```python
from build123d import *

# Parameters (mm, degrees)
BOSS_EXTRUDE1_DEPTH      = 5.5
BOSS_EXTRUDE1_DEPTH_BACK = 5.5
SKETCH2_W                = 108
SKETCH2_H                = 22
CUT_EXTRUDE1_DEPTH       = 11
SKETCH4_W                = 9
SKETCH4_H                = 10
CUT_EXTRUDE2_DEPTH       = 11


with BuildPart() as part:
    # Sketch1 → Boss-Extrude1 (new, two sides: drawn at the far end of the back side and taken through both)
    with BuildSketch(Plane.XY.offset(-BOSS_EXTRUDE1_DEPTH_BACK)):
        with BuildLine():
            Line((0, 0), (27, 0))
            Line((27, 0), (27, 1))
            Line((27, 1), (6.99, 1))
            ThreePointArc((6.99, 1), (6.636446609, 1.146446609), (6.49, 1.5))
            Line((6.49, 1.5), (6.49, 1.724666059))
            Line((6.49, 1.724666059), (4.63, 1.887394973))
            ThreePointArc((4.63, 1.887394973), (5.459499899, 4.491284383), (3.833170563, 6.6875))
            ThreePointArc((3.833170563, 6.6875), (2.5, 4.5), (1.166829437, 6.6875))
            ThreePointArc((1.166829437, 6.6875), (0.515533844, 6.249865346), (0, 5.658312395))
            Line((0, 5.658312395), (0, 0))
        make_face()
    extrude(amount=BOSS_EXTRUDE1_DEPTH + BOSS_EXTRUDE1_DEPTH_BACK)

    # Sketch2 → Cut-Extrude1 (cut)
    with BuildSketch(Plane(origin=(0, 0, 0), x_dir=(1, 0, 0), z_dir=(0, 1, 0))):
        Rectangle(SKETCH2_W, SKETCH2_H)
        with BuildLine():
            Line((0, 5.5), (0, -5.5))
            Line((0, -5.5), (21.5, -5.5))
            ThreePointArc((21.5, -5.5), (27, 0), (21.5, 5.5))
            Line((21.5, 5.5), (0, 5.5))
        make_face(mode=Mode.SUBTRACT)
    extrude(amount=CUT_EXTRUDE1_DEPTH, mode=Mode.SUBTRACT)

    # Sketch4 → Cut-Extrude2 (cut)
    with BuildSketch(Plane(origin=(0, 0, 0), x_dir=(0, 0, -1), z_dir=(1, 0, 0))):
        with Locations((0, 6)):
            Rectangle(SKETCH4_W, SKETCH4_H)
    extrude(amount=CUT_EXTRUDE2_DEPTH, mode=Mode.SUBTRACT)

    # Sketch3 → Cut-Revolve1 (revolve, cut)
    with BuildSketch(Plane.XY, mode=Mode.PRIVATE) as cut_revolve1_sk:
        Polygon((7.5, 1), (9.6, 1), (9.1, 0), (7.5, 0), align=None)
    revolve(cut_revolve1_sk.sketch.rotate(Axis((7.5, 0, 0), (0, 1, 0)), 270), axis=Axis((7.5, 0, 0), (0, 1, 0)), mode=Mode.SUBTRACT)

    # Sketch5 → Cut-Revolve2 (revolve, cut)
    with BuildSketch(Plane.XY, mode=Mode.PRIVATE) as cut_revolve2_sk:
        Polygon((20.5, 1), (22.6, 1), (22.1, 0), (20.5, 0), align=None)
    revolve(cut_revolve2_sk.sketch.rotate(Axis((20.5, 0, 0), (0, 1, 0)), 270), axis=Axis((20.5, 0, 0), (0, 1, 0)), mode=Mode.SUBTRACT)


solid = part.part
```
The model under review builds one solid part; all positions refer to its coordinate system, in mm. A direction names the side the tool comes from. Round coordinates to 2 decimals unless told otherwise and drop trailing zeros. Write each loop counter-clockwise with the first axis right and the second up, starting at its lowest first coordinate (ties: lowest second). Pieces come first, ordered by that corner, then holes.
(1) Wall thickness on L1, parallel to Z at x = 4, y = 1.75; L2, parallel to X at y = 0.75, z = 1.5; L3, parallel to Y at x = 2.5, z = -4.75: over which ranges is each line inside the solid? List them lowest first.
(2) Machinability: for faces 4 (the flat face through (14, 1, 0)), 5 (the flat face through (3, 3, 4.5)), 6 (the flat face through (5.573, 1.805, 4.993)), 7 (the flat face through (5.9, 1.6, 5.5)), 8 (the flat face through (5.9, 1.6, -5.5)), which of the approach directions +Z, -Z, +X, -X, +Y, -Y give a long, thin tool a straight path to every point of the face, cutting with its end or side? Answer none if there is none.
(3) We need section A-A on z = 0. Give the boundary of the cut face in (x, y).
(4) Mouldability with a two-part tool opening along X and no side actions: class faces 1 (the cylindrical face through (27, 0.5, 0.1)), 2 (the cylindrical face through (2.5, 4.5, -5)), 3 (the flat face through (13, 0, 0)) as +X half, -X half, draft (parallel to the pull), parting line (faces both ways), or undercut.
(5) Insertion check: pin 1 (2.5 mm diameter, centred on x = 2.5, y = 6, fed in from -Z); pin 2 (1.5 mm diameter, centred on x = 3, z = -3, fed in from +Y). Each pin has a flat end and moves straight along its axis. Give the tip position at first contact, or say it passes through.
(6) We need section B-B on x = 20.5. Give the boundary of the cut face in (y, z), and give its area (3 significant figures).
(7) We need section D-D on x = 2.5. Give the boundary of the cut face in (y, z).
(8) We need section C-C on y = 2.5. Give the boundary of the cut face in (x, z).
Findings below:
1. L1: z = -5.5 to -4.5, 4.5 to 5.5
1. L2: x = 0 to 6.22, 8.78 to 19.22, 21.78 to 26.79
1. L3: y = 0 to 4.5
2. face 4: +X, +Y
2. face 5: +X, -X, +Y
2. face 6: +Z, -Z, +X
2. face 7: +Z, +X, -X, +Y, -Y
2. face 8: -Z, +X, -X, +Y, -Y
3. outline: (0, 0) - (5.9, 0) - (5.4, 1) - (0, 1) - close; (9.1, 0) - (18.9, 0) - (18.4, 1) - (9.6, 1) - close; (22.1, 0) - (27, 0) - (27, 1) - (22.6, 1) - close
4. face 1: +X half
4. face 2: undercut
4. face 3: draft
5. pin 1: passes through
5. pin 2: stops at y = 1
6. outline: (0, -5.5) - (1, -5.5) - (1, -2.1) - (0, -1.6) - close; (0, 1.6) - (1, 2.1) - (1, 5.5) - (0, 5.5) - close
6. area: 7.30 mm2
7. outline: (0, -5.5) - (4.5, -5.5) - (4.5, -4.5) - (1, -4.5) - (1, 4.5) - (4.5, 4.5) - (4.5, 5.5) - (0, 5.5) - close
8. outline: (0, -5.5) - (5.1, -5.5) - (5.1, -4.5) - (0, -4.5) - close; (0, 4.5) - (5.1, 4.5) - (5.1, 5.5) - (0, 5.5) - close
